Here's how the part is built. I have some questions about the finished solid (model axes, mm). Face numbers are marked on the shaded views. A direction names the side the tool comes from. Round coordinates to 2 decimals unless told otherwise and drop trailing zeros. Write each loop counter-clockwise with the first axis right and the second up, starting at its lowest first coordinate (ties: lowest second). Pieces come first, ordered by that corner, then holes. Notation, with made-up numbers: (10.5, 84.25) -> (64.5, 84.25) arc R22 cw to (64.5, 123.25) -> close; hole circle Ø2 at (-32.75, 9). An arc over 180 degrees is marked (long way). Answer in a Markdown table with one row per item. Add a question column.
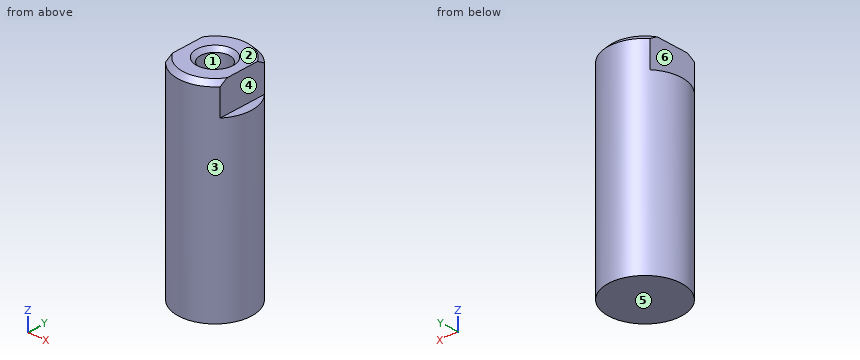
from build123d import *

# Parameters (mm, degrees)
CUT_EXTRUDE_1_DEPTH = 3.4


with BuildPart() as part:
    # 草图1 → 旋转1 (revolve)
    with BuildSketch(Plane(origin=(0, 0, 0), x_dir=(0, 0, -1), z_dir=(1, 0, 0)), mode=Mode.PRIVATE) as revolve_1_sk:
        Polygon((-3.5, 0), (-3.5, 3.5), (-3, 4), (19, 4), (19, 0), align=None)
    revolve(revolve_1_sk.sketch.rotate(Axis((0, 0, -19), (0, 0, 1)), 270), axis=Axis((0, 0, -19), (0, 0, 1)))

    # 草图2 → 切除-拉伸1 (cut)
    with BuildSketch(Plane.XY.offset(3.5)):
        Polygon((-6, -6), (-3, -6), (-3, 6), (3, 6), (3, -6), (6, -6), (6, 8), (-6, 8), align=None)
    extrude(amount=-CUT_EXTRUDE_1_DEPTH, mode=Mode.SUBTRACT)

    # 草图3 → 切除-旋转1 (revolve, cut)
    with BuildSketch(Plane(origin=(0, 0, 0), x_dir=(0, 0, -1), z_dir=(1, 0, 0)), mode=Mode.PRIVATE) as cut_revolve_1_sk:
        Polygon((-4, 0), (-4, 2.5), (-3.07, 1.57), (5, 1.57), (5.906439923, 0), align=None)
    revolve(cut_revolve_1_sk.sketch.rotate(Axis((0, 0, -5.906439923), (0, 0, 1)), 270), axis=Axis((0, 0, -5.906439923), (0, 0, 1)), mode=Mode.SUBTRACT)


solid = part.part
Item 1: I need wall thicknesses on line 1 along Y through (x, z) = (0, 1.25); line 2 along Z through (x, y) = (3.5, 0.25); line 3 along X through (y, z) = (-1.25, -1.5). Which ranges of each line are inside material? Lowest first, please. Write a range as from..to.
Item 2: If we section it at C-C on x = 3.25: Please give me the cut outline in (y, z), then the cut area to 3 significant figures.
Item 3: If we section it at B-B on z = -16: Please give me the cut outline in (x, y).
Item 4: If we mould it in two halves opening along Y, with no side actions, what happens to the marked faces 1, 2 and 3? For each: pulls with the +Y half, pulls with the -Y half, needs draft (parallel to the pull), parting line crosses it, or undercut.
Item 5: For P1, Ø1, axis at y = -1, z = 1, coming from the +X side; P2, Ø3.5, axis at x = 0, y = 0, coming from the +Z side, each with a flat end and sliding along its axis, tell me the tip position at first contact or that it passes through.
Item 6: If we section it at A-A on z = 1.75: Please give me the cut outline in (x, y).
Item 7: On a 3-axis mill with a long thin cutter (end or side, diameter ignored), from which of +Z, -Z, +X, -X, +Y, -Y can I reach the whole of each face in a straight line? I mean the marked faces 4, 5 and 6. Say none if no direction works.
Results list:
| question | item | result |
|---|---|---|
| 1 | line 1 | -4..-1.57, 1.57..4 |
| 1 | line 2 | -19..0.1 |
| 1 | line 3 | -3.8..-0.95, 0.95..3.8 |
| 2 | outline | (-2.33, -19) -> (2.33, -19) -> (2.33, 0.1) -> (-2.33, 0.1) -> close |
| 2 | area | 89.1 mm² |
| 3 | outline | circle Ø8 at (0, 0) |
| 4 | face 1 | undercut |
| 4 | face 2 | needs draft |
| 4 | face 3 | parting line crosses it |
| 5 | P1 | x = 3 |
| 5 | P2 | z = 3.25 |
| 6 | outline | (-3, -2.65) arc R4 ccw to (3, -2.65) -> (3, 2.65) arc R4 ccw to (-3, 2.65) -> close; hole circle Ø3.14 at (0, 0) |
| 7 | face 4 | +Z, +X, +Y, -Y |
| 7 | face 5 | -Z, +X, -X, +Y, -Y |
| 7 | face 6 | +Z, -X, +Y, -Y |
